from build123d import *
from build123d.topology import SkipClean

# Parameters (mm, degrees)
BASE_BLOCK_SKETCH_W   = 60
BASE_BLOCK_SKETCH_H   = 15
BASE_BLOCK_DEPTH      = 25
FORK_UPRIGHT_DEPTH    = 20
ROUNDED_END_LUG_DEPTH = 15
BORE_SKETCH_R         = 15
BORE_30_DEPTH         = 15


with BuildPart() as part:
    # Base Block Sketch → Base Block (new, symmetric)
    with BuildSketch(Plane.XY):
        Rectangle(BASE_BLOCK_SKETCH_W, BASE_BLOCK_SKETCH_H)
    extrude(amount=BASE_BLOCK_DEPTH, both=True)

    # Fork Upright Sketch → Fork Upright (add)
    with BuildSketch(Plane(origin=(30, 0, 0), x_dir=(0, 0, -1), z_dir=(1, 0, 0))):
        Polygon((-20, 7.5), (-20, 37.5), (-12, 37.5), (-12, 17.5), (12, 17.5), (12, 37.5), (20, 37.5), (20, 7.5), align=None)
    extrude(amount=-FORK_UPRIGHT_DEPTH)

    # End Lug Sketch → Rounded End Lug (add)
    with BuildSketch(Plane(origin=(0, 7.5, 0), x_dir=(1, 0, 0), z_dir=(0, 1, 0))):
        with BuildLine():
            Line((-30, 15), (-30, 25))
            ThreePointArc((-30, 25), (-55, 0), (-30, -25))
            Line((-30, -25), (-30, -15))
            ThreePointArc((-30, -15), (-45, 0), (-30, 15))
        make_face()
    extrude(amount=-ROUNDED_END_LUG_DEPTH)

    # Bore Sketch → Bore Ø30 (cut)
    with SkipClean():  # the faces are left unmerged after this step: merging them gives an invalid solid
        with BuildSketch(Plane(origin=(0, 7.5, 0), x_dir=(1, 0, 0), z_dir=(0, 1, 0))):
            with Locations(Location((-30, 0, 0), (0, 0, 270))):
                Circle(BORE_SKETCH_R)
        extrude(amount=-BORE_30_DEPTH, mode=Mode.SUBTRACT)


solid = part.part
For this review, take the finished solid that the model builds, in its own axes (mm). A direction names the side the tool comes from. Coordinates: 2 decimals unless noted, no trailing zeros. Loops run counter-clockwise (first coordinate to the right, second up) from the corner with the lowest first, then second, coordinate; pieces in that order, holes last. Notation, with made-up numbers: (75, 69) - (91, 69) arc R8 ccw to (91, 79) - close; hole circle Ø4 at (-21.5, 38.5). An arc over 180 degrees is marked (long way). Use a Markdown table: item, result. Add a question column.
Item 1: We need section C-C (x = -37). Give the boundary of the cut face in (y, z), and give its area (3 significant figures).
Item 2: We need section A-A (z = 0). Give the boundary of the cut face in (x, y).
Item 3: For line 1 (Z direction, x = -30, y = 0.75); line 2 (X direction, y = 6.5, z = -9); line 3 (X direction, y = 0, z = 0), list the stretches that pass through material, from the lowest coordinate up.
Item 4: We need section D-D (z = 14). Give the boundary of the cut face in (x, y), and give its area (3 significant figures).
Item 5: We need section B-B (y = 0). Give the boundary of the cut face in (x, z).
Item 6: Insertion check: pin 1 Ø6 at (x, y) = (-5, 12) entering from +Z; pin 2 Ø1.5 at (x, y) = (15, 29.5) entering from -Z; pin 3 Ø4 at (y, z) = (13, -1.5) entering from -X; pin 4 Ø16 at (x, y) = (18.5, 26.5) entering from +Z. Each pin has a flat end and moves straight along its axis. Give the tip position at first contact, or say it passes through.
Item 7: Tool access review of faces 1 (the face through (-4, -7.5, 0)), 2 (the face through (10, 16, 0)), 3 (the face through (20, 27, -12)), 4 (the face through (20, 23, -20)), 5 (the face through (20, 22, 20)): name each direction out of +Z, -Z, +X, -X, +Y, -Y from which nothing blocks a thin tool from reaching the whole face with its end or side.
Results list:
| question | item | result |
|---|---|---|
| 1 | outline | (-7.5, -24) - (7.5, -24) - (7.5, -13.27) - (-7.5, -13.27) - close; (-7.5, 13.27) - (7.5, 13.27) - (7.5, 24) - (-7.5, 24) - close |
| 1 | area | 322 mm^2 |
| 2 | outline | (-55, -7.5) - (-45, -7.5) - (-45, 7.5) - (-55, 7.5) - close; (-15, -7.5) - (30, -7.5) - (30, 17.5) - (10, 17.5) - (10, 7.5) - (-15, 7.5) - close |
| 3 | line 1 | z = -25 to -15, 15 to 25 |
| 3 | line 2 | x = -53.32 to -42, -18 to 30 |
| 3 | line 3 | x = -55 to -45, -15 to 30 |
| 4 | outline | (-50.71, -7.5) - (-35.39, -7.5) - (-35.39, 7.5) - (-50.71, 7.5) - close; (-24.61, -7.5) - (30, -7.5) - (30, 37.5) - (10, 37.5) - (10, 7.5) - (-24.61, 7.5) - close |
| 4 | area | 1,650 mm^2 |
| 5 | outline | (-30, -25) - (30, -25) - (30, 25) - (-30, 25) arc R25 ccw to start; hole circle Ø30 at (-30, 0) |
| 6 | pin 1 | passes through |
| 6 | pin 2 | stops at z = -20 |
| 6 | pin 3 | stops at x = 10 |
| 6 | pin 4 | stops at z = 20 |
| 7 | face 1 | +Z, -Z, +X, -X, -Y |
| 7 | face 2 | +Z, -Z, -X, +Y |
| 7 | face 3 | +X, -X, +Y |
| 7 | face 4 | -Z, +X, -X, +Y |
| 7 | face 5 | +Z, +X, -X, +Y |
